Part model, mm, in its own coordinate system. Give positions to 0.01 mm unless a question says otherwise; leave off trailing zeros. Write each loop counter-clockwise with the first axis right and the second up, starting at its lowest first coordinate (ties: lowest second). Pieces come first, ordered by that corner, then holes. Notation, with made-up numbers: M 45,44 L 97,44 A9 ccw 97,60 Z; hole C -27.5,35 d3. An arc over 180 degrees is marked long. Answer as CSV lines item,"result". Start each with the question number.
Item 1: Pin check, flat tip, straight feed: pin 1 (17 mm diameter, centred on x = 0, y = 0, fed in from -Z). Stop position of the tip, or through.
Item 2: Band-saw the part on A-A, the plane z = -0.8. List the corners of the cut face in (x, y).
Item 3: Wall check: L1, parallel to Y at x = 0, z = 0.1; L2, parallel to X at y = -33, z = 0.35; L3, parallel to X at y = -52.5, z = 0.4. Give the ranges that are in metal, low to high. Write a range as from..to.
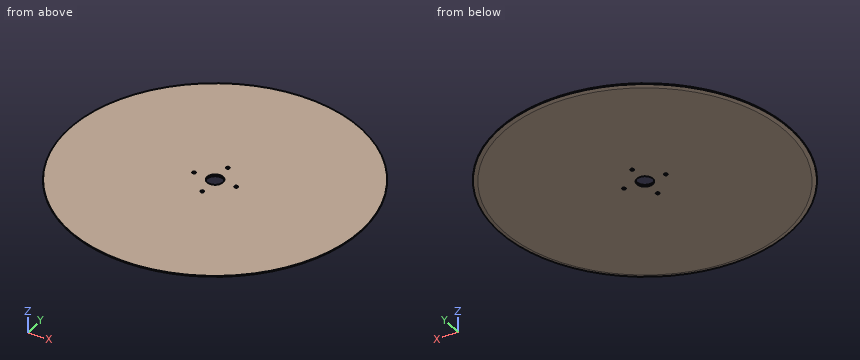
from build123d import *

# Parameters (mm, degrees)
SKETCH_3_R          = 175
EXTRUDE_1_DEPTH     = 1.1
SKETCH_4_R          = 170
EXTRUDE_2_DEPTH     = 1.2
SKETCH_7_R          = 9.5
CUT_EXTRUDE_1_DEPTH = 248.498060598
SKETCH_10_R         = 2
CUT_EXTRUDE_2_DEPTH = 2.3


with BuildPart() as part:
    # 草图3 → 凸台-拉伸1 (new body)
    with BuildSketch(Plane.XY):
        Circle(SKETCH_3_R)
    extrude(amount=EXTRUDE_1_DEPTH)

    # 草图4 → 凸台-拉伸2 (add)
    with BuildSketch(Plane(origin=(0, 0, 0), x_dir=(-1, 0, 0), z_dir=(0, 0, -1))):
        with Locations(Location((0, 0, 0), (0, 0, 180))):
            Circle(SKETCH_4_R)
    extrude(amount=EXTRUDE_2_DEPTH)

    # 草图7 → 切除-拉伸1 (cut, through all)
    with BuildSketch(Plane.XY.offset(1.1)):
        Circle(SKETCH_7_R)
    extrude(amount=-CUT_EXTRUDE_1_DEPTH, mode=Mode.SUBTRACT)

    # 扫描1: sweep along a path in 草图9
    with BuildLine(Plane(origin=(0, 0, 0), x_dir=(-1, 0, 0), z_dir=(0, 0, -1))) as sweep_1_path:
        CenterArc((0, 0), 170, 0, 360)
    # 草图8 → 扫描1 (sweep)
    with BuildSketch(Plane(origin=(0, 0, 0), x_dir=(1, 0, 0), z_dir=(0, 1, 0))):
        Polygon((-175, 0), (-170, 1.2), (-170, 0), align=None)
    sweep(path=sweep_1_path.line)

    # 草图10 → 切除-拉伸2 (cut)
    with BuildSketch(Plane.XY.offset(1.1)):
        with Locations((0, 25)):
            Circle(SKETCH_10_R)
        with Locations((25, 0)):
            Circle(SKETCH_10_R)
        with Locations((0, -25)):
            Circle(SKETCH_10_R)
        with Locations((-25, 0)):
            Circle(SKETCH_10_R)
    extrude(amount=-CUT_EXTRUDE_2_DEPTH, mode=Mode.SUBTRACT)


solid = part.part
Output:
1,pin 1,"through"
2,outline,"C 0,0 d343.33; hole C -25,0 d4; hole C 0,0 d19; hole C 0,-25 d4; hole C 0,25 d4; hole C 25,0 d4"
3,L1,"-175..-27, -23..-9.5, 9.5..23, 27..175"
3,L2,"-171.86..171.86"
3,L3,"-166.94..166.94"
